from build123d import *

# Parameters (mm, degrees)
FRONT_FRAME_DEPTH       = 60
FRAME_MEMBER_2_SKETCH_W = 60
FRAME_MEMBER_2_SKETCH_H = 500
FRAME_MEMBER_2_DEPTH    = 60
FRAME_MEMBER_3_DEPTH    = 60
FRAME_MEMBER_4_DEPTH    = 60
FRAME_MEMBER_5_DEPTH    = 60
FRAME_MEMBER_6_SKETCH_W = 60
FRAME_MEMBER_6_SKETCH_H = 500
FRAME_MEMBER_6_DEPTH    = 60
FRAME_MEMBER_7_DEPTH    = 60
FRAME_MEMBER_8_SKETCH_W = 60
FRAME_MEMBER_8_SKETCH_H = 500
FRAME_MEMBER_8_DEPTH    = 60


with BuildPart() as part:
    # Front Frame Sketch → Front Frame (new body)
    with BuildSketch(Plane.XY):
        Polygon((0, 0), (0, 250), (1000, 250), (1000, 0), (940, 0), (940, 190), (60, 190), (60, 0), align=None)
    extrude(amount=FRONT_FRAME_DEPTH)

    # Frame Member 2 Sketch → Frame Member 2 (add)
    with BuildSketch(Plane(origin=(0, 250, 0), x_dir=(1, 0, 0), z_dir=(0, 1, 0))):
        with Locations((30, 250)):
            Rectangle(FRAME_MEMBER_2_SKETCH_W, FRAME_MEMBER_2_SKETCH_H)
        with Locations((970, 250)):
            Rectangle(FRAME_MEMBER_2_SKETCH_W, FRAME_MEMBER_2_SKETCH_H)
    extrude(amount=-FRAME_MEMBER_2_DEPTH)

    # Frame Member 3 Sketch → Frame Member 3 (add)
    with BuildSketch(Plane(origin=(0, 0, -500), x_dir=(-1, 0, 0), z_dir=(0, 0, -1))):
        Polygon((-1000, 250), (0, 250), (0, 0), (-60, 0), (-60, 190), (-940, 190), (-940, 0), (-1000, 0), align=None)
    extrude(amount=FRAME_MEMBER_3_DEPTH)

    # Frame Member 4 Sketch → Frame Member 4 (add)
    with BuildSketch(Plane.XY.offset(60)):
        Polygon((750, 250), (750, 500), (250, 500), (250, 250), (310, 250), (310, 440), (690, 440), (690, 250), align=None)
    extrude(amount=-FRAME_MEMBER_4_DEPTH)

    # Frame Member 5 Sketch → Frame Member 5 (add)
    with BuildSketch(Plane(origin=(0, 0, -560), x_dir=(-1, 0, 0), z_dir=(0, 0, -1))):
        Polygon((-750, 250), (-750, 500), (-250, 500), (-250, 250), (-310, 250), (-310, 440), (-690, 440), (-690, 250), align=None)
    extrude(amount=-FRAME_MEMBER_5_DEPTH)

    # Frame Member 6 Sketch → Frame Member 6 (add)
    with BuildSketch(Plane(origin=(0, 250, 0), x_dir=(1, 0, 0), z_dir=(0, 1, 0))):
        with Locations((280, 250)):
            Rectangle(FRAME_MEMBER_6_SKETCH_W, FRAME_MEMBER_6_SKETCH_H)
        with Locations((720, 250)):
            Rectangle(FRAME_MEMBER_6_SKETCH_W, FRAME_MEMBER_6_SKETCH_H)
    extrude(amount=-FRAME_MEMBER_6_DEPTH)

    # Frame Member 7 Sketch → Frame Member 7 (add)
    with BuildSketch(Plane(origin=(0, 250, 0), x_dir=(1, 0, 0), z_dir=(0, 1, 0))):
        Polygon((310, 250), (310, 280), (690, 280), (690, 220), (310, 220), align=None)
    extrude(amount=-FRAME_MEMBER_7_DEPTH)

    # Frame Member 8 Sketch → Frame Member 8 (add)
    with BuildSketch(Plane(origin=(0, 500, 0), x_dir=(1, 0, 0), z_dir=(0, 1, 0))):
        with Locations((405, 250)):
            Rectangle(FRAME_MEMBER_8_SKETCH_W, FRAME_MEMBER_8_SKETCH_H)
        with Locations((595, 250)):
            Rectangle(FRAME_MEMBER_8_SKETCH_W, FRAME_MEMBER_8_SKETCH_H)
    extrude(amount=-FRAME_MEMBER_8_DEPTH)


solid = part.part
The model under review builds one solid part; all positions refer to its coordinate system, in mm. A direction names the side the tool comes from. Coordinates: 2 decimals unless noted, no trailing zeros. Write each loop counter-clockwise with the first axis right and the second up, starting at its lowest first coordinate (ties: lowest second). Pieces come first, ordered by that corner, then holes. Notation, with made-up numbers: (42.25, 68) -> (69.25, 68) arc R28 cw to (69.25, 95) -> close; hole circle Ø7 at (-2, 85). An arc over 180 degrees is marked (long way). Answer in a Markdown table with one row per item.
1. Clearance check with flat-ended pins moving along their axes: pin 1 Ø12 at (x, z) = (287, -49.5) entering from -Y; pin 2 Ø18 at (y, z) = (299, 25.5) entering from +X. State where each tip first meets the part, or that it passes through.
Answers below:
| item | result |
|---|---|
| pin 1 | stops at y = 190 |
| pin 2 | stops at x = 750 |
2. Draft analysis for pull direction X (two halves, no side actions). For faces 4 (the flat face through (503, 220, -220)), 5 (the flat face through (1000, 207, -246)), 6 (the flat face through (970, 0, 30)), state which applies: +X half, -X half, draft (parallel to the pull), parting line (faces both ways), or undercut.
Answers below:
| item | result |
|---|---|
| face 4 | undercut |
| face 5 | +X half |
| face 6 | draft |
3. We need section A-A, the plane z = -142.5. State the section outline as (x, y) points.
Answers below:
| item | result |
|---|---|
| outline | (0, 190) -> (60, 190) -> (60, 250) -> (0, 250) -> close; (250, 190) -> (310, 190) -> (310, 250) -> (250, 250) -> close; (375, 440) -> (435, 440) -> (435, 500) -> (375, 500) -> close; (565, 440) -> (625, 440) -> (625, 500) -> (565, 500) -> close; (690, 190) -> (750, 190) -> (750, 250) -> (690, 250) -> close; (940, 190) -> (1000, 190) -> (1000, 250) -> (940, 250) -> close |
4. Wall thickness on probe 1 along Z at (x, y) = (395.5, 196); probe 2 along X at (y, z) = (204, -422.5); probe 3 along X at (y, z) = (357.5, -506.5): over which ranges is each line inside the solid? List them lowest first. Write a range as [from, to].
Answers below:
| item | result |
|---|---|
| probe 1 | z = [-560, -500], [-280, -220], [0, 60] |
| probe 2 | x = [0, 60], [250, 310], [690, 750], [940, 1000] |
| probe 3 | x = [250, 310], [690, 750] |
5. For faces 1 (the flat face through (286, 405, 0)), 2 (the flat face through (154, 220, -500)), 3 (the flat face through (310, 344, 30)), list the 3-axis set-ups (+Z, -Z, +X, -X, +Y, -Y) from which the entire face can be reached by the end or side of a thin tool; tool diameter is ignored.
Answers below:
| item | result |
|---|---|
| face 1 | -X, +Y |
| face 2 | +Y, -Y |
| face 3 | +Z, -Z |
6. We need section B-B, the plane y = 73. State the section outline as (x, z) points, and give its area (3 significant figures).
Answers below:
| item | result |
|---|---|
| outline | (0, -560) -> (60, -560) -> (60, -500) -> (0, -500) -> close; (0, 0) -> (60, 0) -> (60, 60) -> (0, 60) -> close; (940, -560) -> (1000, -560) -> (1000, -500) -> (940, -500) -> close; (940, 0) -> (1000, 0) -> (1000, 60) -> (940, 60) -> close |
| area | 14,400 mm^2 |
7. We need section C-C, the plane x = 230.5. State the section outline as (y, z) points.
Answers below:
| item | result |
|---|---|
| outline | (190, -560) -> (250, -560) -> (250, -500) -> (190, -500) -> close; (190, 0) -> (250, 0) -> (250, 60) -> (190, 60) -> close |
8. We need section D-D, the plane z = -520.5. State the section outline as (x, y) points.
Answers below:
| item | result |
|---|---|
| outline | (0, 0) -> (60, 0) -> (60, 190) -> (940, 190) -> (940, 0) -> (1000, 0) -> (1000, 250) -> (750, 250) -> (750, 500) -> (250, 500) -> (250, 250) -> (0, 250) -> close; hole (310, 250) -> (690, 250) -> (690, 440) -> (310, 440) -> close |
